Geometry check sheet. Reference: the model listing, model coordinates, mm. A direction names the side the tool comes from. Coordinates: 2 decimals unless noted, no trailing zeros. Write each loop counter-clockwise with the first axis right and the second up, starting at its lowest first coordinate (ties: lowest second). Pieces come first, ordered by that corner, then holes. Notation, with made-up numbers: (-19.75, 76.5) -> (21.25, 76.5) arc R9 cw to (21.25, 83.5) -> close; hole circle Ø3 at (41, 38.5). An arc over 180 degrees is marked (long way). One line per question, with ' | ' between items.
from build123d import *

# Parameters (mm, degrees)
SKETCH1_W           = 57
SKETCH1_H           = 57
BOSS_EXTRUDE1_DEPTH = 51
SKETCH2_R           = 2.5
CUT_EXTRUDE1_DEPTH  = 98
SKETCH4_R           = 10
BOSS_EXTRUDE2_DEPTH = 1
SKETCH5_R           = 4
BOSS_EXTRUDE3_DEPTH = 21
CUT_EXTRUDE2_DEPTH  = 21


with BuildPart() as part:
    # Sketch1 → Boss-Extrude1 (new body)
    with BuildSketch(Plane.XY):
        Rectangle(SKETCH1_W, SKETCH1_H)
    extrude(amount=BOSS_EXTRUDE1_DEPTH)

    # Sketch2 → Cut-Extrude1 (cut)
    with BuildSketch(Plane.XY.offset(51)):
        with Locations((-23.5, 23.5)):
            Circle(SKETCH2_R)
        with Locations((23.5, 23.5)):
            Circle(SKETCH2_R)
        with Locations((23.5, -23.5)):
            Circle(SKETCH2_R)
        with Locations((-23.5, -23.5)):
            Circle(SKETCH2_R)
    extrude(amount=-CUT_EXTRUDE1_DEPTH, mode=Mode.SUBTRACT)

    # Sketch4 → Boss-Extrude2 (add)
    with BuildSketch(Plane.XY.offset(51)):
        Circle(SKETCH4_R)
    extrude(amount=BOSS_EXTRUDE2_DEPTH)

    # Sketch5 → Boss-Extrude3 (add)
    with BuildSketch(Plane.XY.offset(52)):
        with Locations(Location((0, 0, 0), (0, 0, 180))):
            Circle(SKETCH5_R)
    extrude(amount=BOSS_EXTRUDE3_DEPTH)

    # Sketch6 → Cut-Extrude2 (cut)
    with BuildSketch(Plane.XY.offset(73)):
        Polygon((3, 101.241638907), (3, 2.645751311), (3, -2.645751311), (3, -101.241638907), (200.191775192, -101.241638907), (200.191775192, 101.241638907), align=None)
    extrude(amount=-CUT_EXTRUDE2_DEPTH, mode=Mode.SUBTRACT)


solid = part.part
1. Cross-section at D-D on x = 0. Record the boundary of the cut face in (y, z).
Worked answers:
outline: (-28.5, 0) -> (28.5, 0) -> (28.5, 51) -> (10, 51) -> (10, 52) -> (4, 52) -> (4, 73) -> (-4, 73) -> (-4, 52) -> (-10, 52) -> (-10, 51) -> (-28.5, 51) -> close
2. Go/stop test with flat-tipped pins: P1, Ø8, axis at x = 23.5, y = 23.5, coming from the +Z side; P2, Ø4, axis at y = -0.5, z = 66.5, coming from the +X side; P3, Ø4, axis at x = -20, y = 22, coming from the -Z side. Record where each tip stops, or that it passes through.
Worked answers:
P1: z = 51 | P2: x = 3 | P3: z = 0
3. Mould release check, pull along Y, two halves, no side actions. Record for faces 3 (the face through (-25.34, -21.81, 25.86)), 4 (the face through (21.66, -21.81, 25.86)), 5 (the face through (0, -28.5, 25)), 6 (the face through (3, 0, 63)): released by +Y, released by -Y, zero draft, split by the parting line, or undercut.
Worked answers:
face 3: undercut | face 4: undercut | face 5: released by -Y | face 6: zero draft
4. Cross-section at B-B on z = 20. Record the boundary of the cut face in (x, y).
Worked answers:
outline: (-28.5, -28.5) -> (28.5, -28.5) -> (28.5, 28.5) -> (-28.5, 28.5) -> close; hole circle Ø5 at (-23.5, -23.5); hole circle Ø5 at (-23.5, 23.5); hole circle Ø5 at (23.5, -23.5); hole circle Ø5 at (23.5, 23.5)
5. Cross-section at A-A on y = 23.5. Record the boundary of the cut face in (x, z), and give its area (3 significant figures).
Worked answers:
outline: (-28.5, 0) -> (-26, 0) -> (-26, 51) -> (-28.5, 51) -> close; (-21, 0) -> (21, 0) -> (21, 51) -> (-21, 51) -> close; (26, 0) -> (28.5, 0) -> (28.5, 51) -> (26, 51) -> close | area: 2,400 mm²
6. Material ranges on line 1 (Y direction, x = -23.5, z = 20); line 2 (Y direction, x = -23, z = 25); line 3 (Z direction, x = -0.5, y = 13.5), recorded low to high. Write a range as from..to.
Worked answers:
line 1: -28.5..-26, -21..21, 26..28.5 | line 2: -28.5..-25.95, -21.05..21.05, 25.95..28.5 | line 3: 0..51
7. Tool access check on faces 1 (the face through (-4, 0, 62)), 2 (the face through (0, 0, 73)). Record the directions out of +Z, -Z, +X, -X, +Y, -Y that give a thin tool (end or side, any length) a straight path to the whole face; none if there is none.
Worked answers:
face 1: +Z | face 2: +Z, +X, -X, +Y, -Y
